```python
from build123d import *

# Parameters (mm, degrees)
EXTRUDE_1_DEPTH         = 110
CUT_EXTRUDE_1_DEPTH     = 156.879643007
HOLE_WIZARD_11_0_11_1_D = 11
CHAMFER_1_SIZE          = 5
FILLET_1_R              = 8
FILLET_2_R              = 16


with BuildPart() as part:
    # 草图1 → 凸台-拉伸1 (new body)
    with BuildSketch(Plane.XY.offset(110)):
        Polygon((50, 0), (50, 92.726312153), (17.364817767, 98.480775301), (0, 0), align=None)
    extrude(amount=-EXTRUDE_1_DEPTH)

    # 草图2 → 切除-拉伸1 (cut, through all)
    with BuildSketch(Plane(origin=(0, 0, 0), x_dir=(-1, 0, 0), z_dir=(0, 0, -1))):
        Polygon((-9.534028741, 8), (-25.243279791, 97.09158988), (-50, 92.726312153), (-50, 8), align=None)
    extrude(amount=-CUT_EXTRUDE_1_DEPTH, mode=Mode.SUBTRACT)

    # Ø11.0 (11) 直径孔1 (through all)
    with Locations(Plane(origin=(0, 8, 0), x_dir=(1, 0, 0), z_dir=(0, 1, 0))):
        with Locations((35, -15), (35, -95)):
            Hole(HOLE_WIZARD_11_0_11_1_D / 2)

    # 倒角1
    chamfer_1_edges = [part.edges().sort_by_distance(p)[0] for p in [
        (50, 4, 110),
        (50, 4, 0),
    ]]
    chamfer(chamfer_1_edges, length=CHAMFER_1_SIZE)

    # 圆角1
    fillet_1_edges = [part.edges().sort_by_distance(p)[0] for p in [
        (9.534028741, 8, 55),
    ]]
    fillet(fillet_1_edges, radius=FILLET_1_R)

    # 圆角2
    fillet_2_edges = [part.edges().sort_by_distance(p)[0] for p in [
        (0, 0, 55),
    ]]
    fillet(fillet_2_edges, radius=FILLET_2_R)


solid = part.part
```
Can you work these out from the model? Positions are in its coordinate system, mm. A direction names the side the tool comes from. Give positions to 0.01 mm unless a question says otherwise; leave off trailing zeros. Loops run counter-clockwise (first coordinate to the right, second up) from the corner with the lowest first, then second, coordinate; pieces in that order, holes last. Notation, with made-up numbers: M 12.25,43.5 L 40.25,43.5 A18 ccw 40.25,47.5 Z; hole C 88.25,11.25 d7. An arc over 180 degrees is marked long. Use CSV: the item, a comma, the result in double quotes. Start each with the question number.
1. If I drill on L1, parallel to Z at x = 35, y = 3.25; L2, parallel to Y at x = 28.5, z = 94; L3, parallel to X at y = 2, z = 95, over which ranges is the centre line in solid material (lowest first)?
2. On a 3-axis mill with a long thin cutter (end or side, diameter ignored), from which of +Z, -Z, +X, -X, +Y, -Y can I reach the whole of each face in a straight line? I mean faces 1 (the face through (10.436, 59.187, 55.77)), 2 (the face through (35, 8, 54)). Say none if no direction works.
3. For P1, Ø3, axis at x = 8, z = 53.5, coming from the -Y side; P2, Ø12, axis at y = 78, z = 86, coming from the +X side; P3, Ø2, axis at x = 28, z = 28, coming from the +Y side, each with a flat end and sliding along its axis, tell me the tip position at first contact or that it passes through.
4. Imagine slicing it at A-A, the plane z = 15. Write out the boundary of the cut face in (x, y), plus the area to 3 significant figures.
5. Imagine slicing it at D-D, the plane z = 80. Write out the boundary of the cut face in (x, y), plus the area to 3 significant figures.
6. Imagine slicing it at B-B, the plane x = 35. Write out the boundary of the cut face in (y, z), plus the area to 3 significant figures.
7. Imagine slicing it at C-C, the plane x = 14. Write out the boundary of the cut face in (y, z), plus the area to 3 significant figures.
8. If we mould it in two halves opening along Y, with no side actions, what happens to faces 3 (the face through (18.118, 56.682, 54.23)), 4 (the face through (21.359, 97.776, 55.77)), 5 (the face through (34, 0, 56))? For each: released by +Y, released by -Y, zero draft, split by the parting line, or undercut.
Response values:
1,L1,"0 to 9.5, 20.5 to 89.5, 100.5 to 110"
1,L2,"0 to 8"
1,L3,"11.32 to 29.5, 40.5 to 50"
2,face 1,"+Z, -Z, -X, +Y"
2,face 2,"+Z, -Z, +X"
3,P1,"y = 3.18"
3,P2,"x = 22.93"
3,P3,"y = 8"
4,outline,"M 3.31,18.78 A16 ccw 19.07,0 L 29.5,0 L 29.5,8 L 19.07,8 A8 cw 11.19,17.39 L 25.24,97.09 L 17.36,98.48 Z; M 40.5,0 L 50,0 L 50,8 L 40.5,8 Z"
4,area,"974 mm^2"
5,outline,"M 3.31,18.78 A16 ccw 19.07,0 L 50,0 L 50,8 L 19.07,8 A8 cw 11.19,17.39 L 25.24,97.09 L 17.36,98.48 Z"
5,area,"1,060 mm^2"
6,outline,"M 0,0 L 8,0 L 8,9.5 L 0,9.5 Z; M 0,20.5 L 8,20.5 L 8,89.5 L 0,89.5 Z; M 0,100.5 L 8,100.5 L 8,110 L 0,110 Z"
6,area,"704 mm^2"
7,outline,"M 0.82,0 L 9.81,0 L 9.81,110 L 0.82,110 Z; M 33.33,0 L 79.4,0 L 79.4,110 L 33.33,110 Z"
7,area,"6,060 mm^2"
8,face 3,"undercut"
8,face 4,"released by +Y"
8,face 5,"released by -Y"
